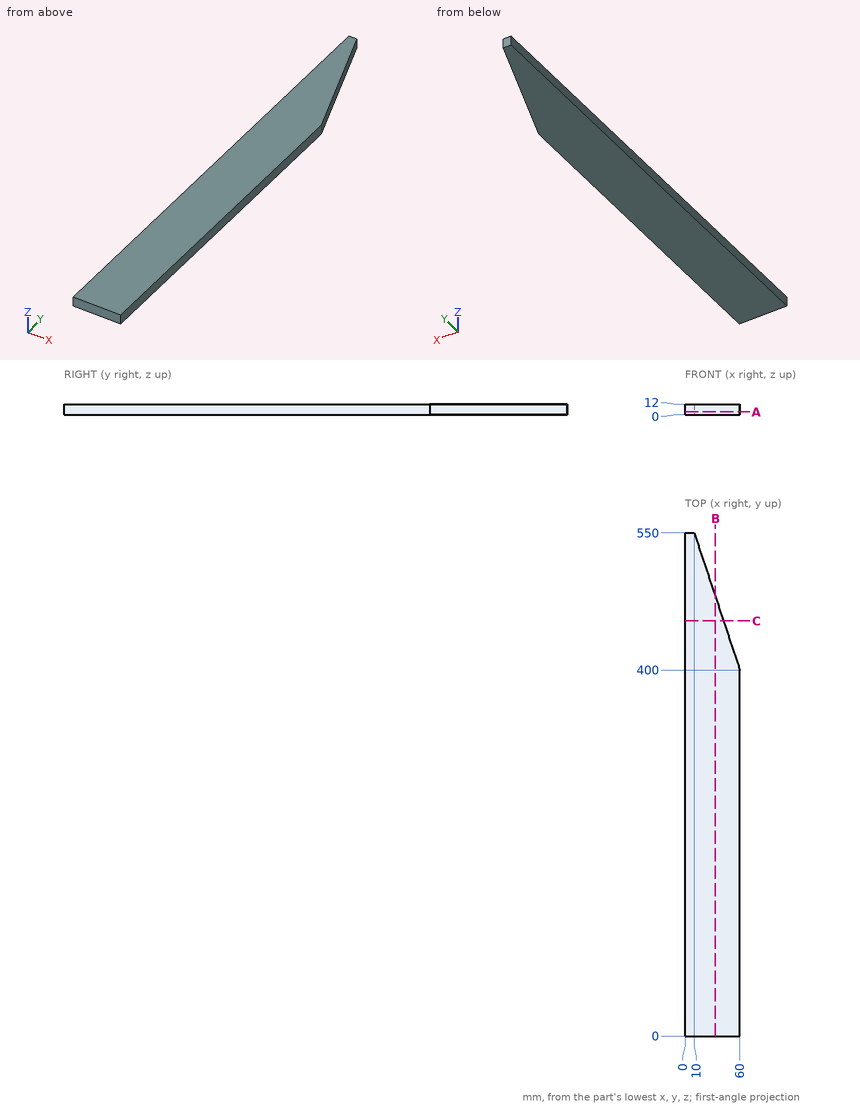
Can you work these out from the drawing? Everything is in mm from the part's minimum corner. Give positions to 0.01 mm unless a question says otherwise; leave off trailing zeros. Loops run counter-clockwise (first coordinate to the right, second up) from the corner with the lowest first, then second, coordinate; pieces in that order, holes last. Notation, with made-up numbers: (15.25, 26.25) -> (44.25, 26.25) arc R22 cw to (44.25, 37.25) -> close; hole circle Ø8 at (45, -9). An arc over 180 degrees is marked (long way). Return JSON: item names as keys, results as strings.
Item 1: I'm going to push a flat-ended pin straight in: pin 1 (1.5 mm diameter, centred on y = 421, z = 6, fed in from +X). Where does the tip first touch, or does it pass through?
Geometry results:
{"pin 1": "stops at x = 53.25"}
Item 2: I need wall thicknesses on L1, parallel to X at y = 475, z = 11; L2, parallel to X at y = 515.5, z = 0.5. Which ranges of each line are inside material? Lowest first, please. Write a range as from..to.
Geometry results:
{"L1": "x = 0..35", "L2": "x = 0..21.5"}
Item 3: If we section it at C-C on y = 454: List the corners of the cut face in (x, z) for me.
Geometry results:
{"outline": "(0, 0) -> (42, 0) -> (42, 12) -> (0, 12) -> close"}
Item 4: If we section it at B-B on x = 33: List the corners of the cut face in (y, z) for me.
Geometry results:
{"outline": "(0, 0) -> (481, 0) -> (481, 12) -> (0, 12) -> close"}
Item 5: If we section it at A-A on z = 3.5: List the corners of the cut face in (x, y) for me.
Geometry results:
{"outline": "(0, 0) -> (60, 0) -> (60, 400) -> (10, 550) -> (0, 550) -> close"}
